from build123d import *

# Parameters (mm, degrees)
CHAMFER_1_SIZE           = 0.5
PATTERN_CIRCULAR_1_COUNT = 4


with BuildPart() as part:
    # 草图2 → 旋转1 (revolve)
    with BuildSketch(Plane.XY, mode=Mode.PRIVATE) as revolve_1_sk:
        Polygon((0, 0), (0, 40), (10, 40), (10, 13), (12, 13), (12, 14), (40, 14), (40, 0), align=None)
    revolve(revolve_1_sk.sketch.rotate(Axis((0, 0, 0), (1, 0, 0)), 90), axis=Axis((0, 0, 0), (1, 0, 0)))

    # 倒角1
    chamfer_1_edges = [part.edges().sort_by_distance(p)[0] for p in [
        (40, 0, -14),
        (10, 0, -40),
        (0, 0, -40),
    ]]
    chamfer(chamfer_1_edges, length=CHAMFER_1_SIZE)

    # 草图7 → 打孔尺寸(%根据)内六角圆柱头螺钉的类型1 (revolve, cut)
    with BuildSketch(Plane(origin=(10, 30, 0), x_dir=(0, 0, -1), z_dir=(0, 1, 0))):
        Polygon((0, 0), (0, 13.152366702), (2.75, 11.5), (2.75, 5.7), (5, 5.7), (5, 0), align=None)
    hole_wizard_1 = revolve(axis=Axis((16.35, 30, 0), (-1, 0, 0)), mode=Mode.SUBTRACT)

    # 阵列(圆周)1: 打孔尺寸(%根据)内六角圆柱头螺钉的类型1 ×4 about axis
    pattern_circular_1_axis = Axis((0, 0, 0), (1, 0, 0))
    for i in range(1, PATTERN_CIRCULAR_1_COUNT):
        add(hole_wizard_1.rotate(pattern_circular_1_axis, i * 360 / PATTERN_CIRCULAR_1_COUNT), mode=Mode.SUBTRACT)


solid = part.part
For this review, take the finished solid that the model builds, in its own axes (mm). A direction names the side the tool comes from. Round coordinates to 2 decimals unless told otherwise and drop trailing zeros. Write each loop counter-clockwise with the first axis right and the second up, starting at its lowest first coordinate (ties: lowest second). Pieces come first, ordered by that corner, then holes. Notation, with made-up numbers: (-4.75, -24.75) -> (31.25, -24.75) arc R13 cw to (31.25, -4.75) -> close; hole circle Ø11 at (83.5, 66). An arc over 180 degrees is marked (long way). Use CSV: the item, a comma, the result in double quotes.
(1) Draft analysis for pull direction X (two halves, no side actions). For faces 1 (the face through (4.3, -32.2, -2.2)), 2 (the face through (11.014, 7.91, -10.316)), 3 (the face through (7.19, 1.08, -34.88)), state which applies: +X half, -X half, draft (parallel to the pull), parting line (faces both ways), or undercut.
Computed values:
face 1,"+X half"
face 2,"undercut"
face 3,"draft"
(2) Consider section C-C, the plane x = 26.5. Give the boundary of the cut face in (y, z).
Computed values:
outline,"circle Ø28 at (0, 0)"
(3) For faces 4 (the face through (4.3, 2.2, -32.2)), 5 (the face through (12, 9.3, -9.3)), 6 (the face through (2.18, 27.273, 0.358)), list the 3-axis set-ups (+Z, -Z, +X, -X, +Y, -Y) from which the entire face can be reached by the end or side of a thin tool; tool diameter is ignored.
Computed values:
face 4,"+X"
face 5,"none"
face 6,"+X, -X"
(4) Consider section A-A, the plane y = 0. Give the number of separate pieces and of enclosed holes in the cut face, plus the area to 3 significant figures.
Computed values:
separate pieces,"3"
enclosed holes,"0"
area,"1,470 mm²"
(5) Clearance check with flat-ended pins moving along their axes: P1, Ø11, axis at y = 0, z = -27.5, coming from the +X side; P2, Ø10, axis at x = 8, z = 16, coming from the +Y side; P3, Ø8, axis at y = 0, z = -30, coming from the +X side. State where each tip first meets the part, or that it passes through.
Computed values:
P1,"x = 10"
P2,"y = 38.46"
P3,"x = 4.3"
(6) To check wall thickness, follow L1, parallel to Y at x = 8.05, z = 0; L2, parallel to X at y = 26.5, z = 25; L3, parallel to Y at x = 17, z = 0.5. State the ranges of each line that lie inside material, in increasing order. Write a range as [from, to].
Computed values:
L1,"[-40, -35], [-25, 25], [35, 40]"
L2,"[0, 10]"
L3,"[-13.99, 13.99]"
